Part model, mm, in its own coordinate system. Face numbers are marked on the shaded views. A direction names the side the tool comes from. Coordinates: 2 decimals unless noted, no trailing zeros. Order: outer loops, then holes, each group sorted by start corner. A loop starts at its lowest first (then second) coordinate and runs counter-clockwise, first axis right, second up.
1) Pin check, flat tips, straight feed: pin 1 Ø1.2 at (x, z) = (2.5, 0) entering from -Y; pin 2 Ø3 at (x, y) = (60.5, 2.5) entering from +Z. Stop position of each tip, or through.
2) Cut at C-C (x = 2.5). List the corners of the cut face in (y, z), and give its area (3 significant figures).
3) Cut at D-D (x = 58). List the corners of the cut face in (y, z).
4) Cut at A-A (y = 0). List the corners of the cut face in (x, z).
5) Cut at B-B (z = 0). Give the number of separate pieces and of enclosed holes in the cut face, and give its area (3 significant figures).
6) Wall check: L1, parallel to X at y = 0.25, z = 0; L2, parallel to X at y = -1, z = -4; L3, parallel to Y at x = 16, z = 0. Give the ranges that are in metal, low to high.
7) Tool access for the marked faces 1, 2 and 3: list every direction of +Z, -Z, +X, -X, +Y, -Y with a clear straight run to the whole face (end or side of a thin tool).
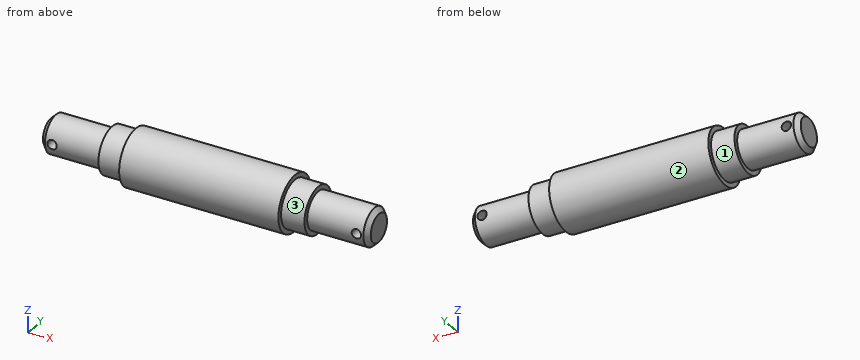
```python
from build123d import *

# Parameters (mm, degrees)
CROSS_HOLE_2_END_1_SKETCH_R = 1
CROSS_HOLE_2_END_1_DEPTH    = 5
CROSS_HOLE_2_END_2_SKETCH_R = 1
CROSS_HOLE_2_END_2_DEPTH    = 11.5
END_CHAMFER_1X45_SIZE       = 1


with BuildPart() as part:
    # Shaft Profile Sketch → Stepped Shaft Body (revolve)
    with BuildSketch(Plane.XY, mode=Mode.PRIVATE) as stepped_shaft_body_sk:
        Polygon((0, 0), (70, 0), (70, -4), (57, -4), (57, -5), (52, -5), (52, -6), (18, -6), (18, -5), (13, -5), (13, -4), (0, -4), align=None)
    revolve(stepped_shaft_body_sk.sketch.rotate(Axis((0, 0, 0), (1, 0, 0)), 270), axis=Axis((0, 0, 0), (1, 0, 0)))

    # Cross Hole Ø2 End 1 Sketch → Cross Hole Ø2 End 1 (cut, symmetric)
    with BuildSketch(Plane(origin=(0, 0, 0), x_dir=(1, 0, 0), z_dir=(0, 1, 0))):
        with Locations(Location((2.5, 0, 0), (0, 0, 270))):
            Circle(CROSS_HOLE_2_END_1_SKETCH_R)
    extrude(amount=CROSS_HOLE_2_END_1_DEPTH, both=True, mode=Mode.SUBTRACT)

    # Cross Hole Ø2 End 2 Sketch → Cross Hole Ø2 End 2 (cut, symmetric)
    with BuildSketch(Plane(origin=(0, 0, 0), x_dir=(1, 0, 0), z_dir=(0, 1, 0))):
        with Locations(Location((67.5, 0, 0), (0, 0, 270))):
            Circle(CROSS_HOLE_2_END_2_SKETCH_R)
    extrude(amount=CROSS_HOLE_2_END_2_DEPTH, both=True, mode=Mode.SUBTRACT)

    # End Chamfer 1x45°
    end_chamfer_1x45_edges = [part.edges().sort_by_distance(p)[0] for p in [
        (70, 0, -4),
        (0, 0, -4),
    ]]
    chamfer(end_chamfer_1x45_edges, length=END_CHAMFER_1X45_SIZE)


solid = part.part
```
Geometry check:
1. pin 1: passes through
1. pin 2: stops at z = 3.87
2. outline: (-3.87, -1) arc R4 ccw to (3.87, -1) - close; (-3.87, 1) - (3.87, 1) arc R4 ccw to start
2. area: 34.4 mm2
3. outline: circle Ø8 at (0, 0)
4. outline: (0, -3) - (1, -4) - (13, -4) - (13, -5) - (18, -5) - (18, -6) - (52, -6) - (52, -5) - (57, -5) - (57, -4) - (69, -4) - (70, -3) - (70, 3) - (69, 4) - (57, 4) - (57, 5) - (52, 5) - (52, 6) - (18, 6) - (18, 5) - (13, 5) - (13, 4) - (1, 4) - (0, 3) - close; hole circle Ø2 at (2.5, 0); hole circle Ø2 at (67.5, 0)
5. separate pieces: 3
5. enclosed holes: 0
5. area: 682 mm2
6. L1: x = 0 to 1.5, 3.5 to 66.5, 68.5 to 70
6. L2: x = 13 to 57
6. L3: y = -5 to 5
7. face 1: -X
7. face 2: +X, -X
7. face 3: +X
